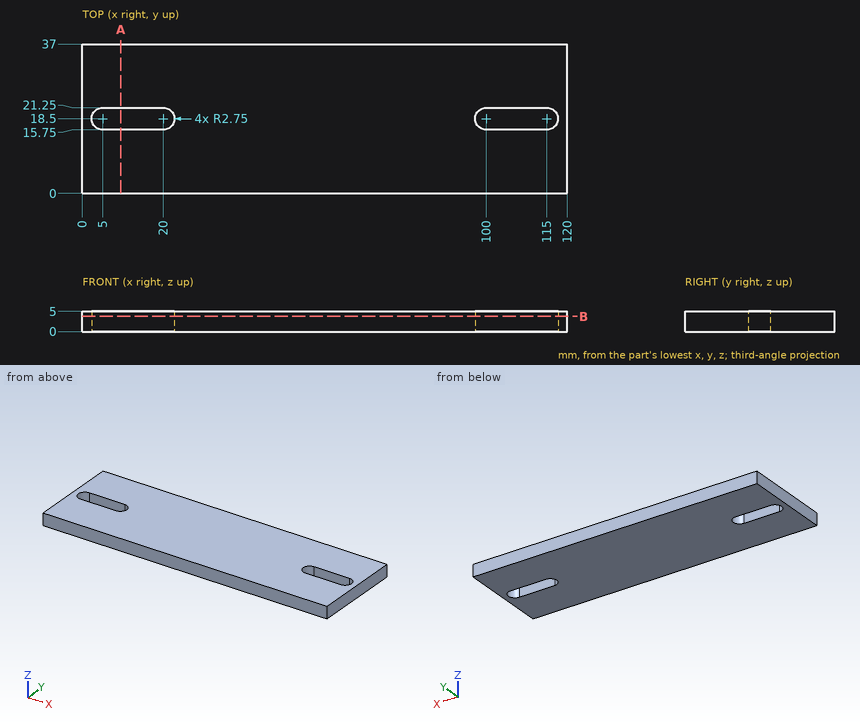
Print and shaded views of the part. All mm, measured from the part's lowest x, y and z. Round coordinates to 2 decimals unless told otherwise and drop trailing zeros. Write each loop counter-clockwise with the first axis right and the second up, starting at its lowest first coordinate (ties: lowest second). Pieces come first, ordered by that corner, then holes. Notation, with made-up numbers: (-29, 34.5) - (8, 34.5) arc R14 ccw to (8, 38.5) - close; hole circle Ø6 at (41, 15). An arc over 180 degrees is marked (long way). Write each question's results on one line, items separated by ' | '. Start each with the question number.
Item 1: Saw through at A-A (x = 9.5). Write the cut outline in (y, z).
Item 2: Saw through at B-B (z = 3.8). Write the cut outline in (x, y).
Item 3: Wall check: L1, parallel to X at y = 17.5, z = 3.2; L2, parallel to Y at x = 113, z = 4.15; L3, parallel to X at y = 16.5, z = 4.75. Give the ranges that are in metal, low to high. Write a range as [from, to].
Results are:
1) outline: (0, 0) - (15.75, 0) - (15.75, 5) - (0, 5) - close; (21.25, 0) - (37, 0) - (37, 5) - (21.25, 5) - close
2) outline: (0, 0) - (120, 0) - (120, 37) - (0, 37) - close; hole (5, 15.75) - (20, 15.75) arc R2.75 ccw to (20, 21.25) - (5, 21.25) arc R2.75 ccw to start; hole (100, 15.75) - (115, 15.75) arc R2.75 ccw to (115, 21.25) - (100, 21.25) arc R2.75 ccw to start
3) L1: x = [0, 2.44], [22.56, 97.44], [117.56, 120] | L2: y = [0, 15.75], [21.25, 37] | L3: x = [0, 3.11], [21.89, 98.11], [116.89, 120]
